Can you work these out from the model? Positions are in its coordinate system, mm. Face numbers are marked on the shaded views. A direction names the side the tool comes from. Coordinates: 2 decimals unless noted, no trailing zeros. Write each loop counter-clockwise with the first axis right and the second up, starting at its lowest first coordinate (ties: lowest second). Pieces come first, ordered by that corner, then holes. Notation, with made-up numbers: (-29.5, 63) - (-4.5, 63) arc R25 cw to (-4.5, 95) - close; hole circle Ø2 at (17, 69.5). An arc over 180 degrees is marked (long way). Write each question's results on one line, items separated by ' | '. Start each with the question number.
```python
from build123d import *

# Parameters (mm, degrees)
BASE_PROFILE_SKETCH_R       = 12.5
BASE_PROFILE_SKETCH_R_2     = 7.5
BASE_PLATE_DEPTH            = 15
SKETCH1_3_W                 = 30
SKETCH1_3_H                 = 15
LOWER_LUG_DEPTH             = 45
LOWER_LUG_CUT_SKETCH_R      = 6
LOWER_LUG_PROFILE_CUT_DEPTH = 45
UPRIGHT_LUG_SKETCH_R        = 6
UPRIGHT_LUG_12_HOLE_DEPTH   = 15


with BuildPart() as part:
    # Base Profile Sketch → Base Plate (new body)
    with BuildSketch(Plane(origin=(0, 0, 0), x_dir=(1, 0, 0), z_dir=(0, 1, 0))):
        with BuildLine():
            Line((150, 25), (0, 25))
            ThreePointArc((0, 25), (-25, 0), (0, -25))
            Line((0, -25), (102.111825559, -25))
            Line((102.111825559, -25), (120, -25))
            Line((120, -25), (150, -25))
            Line((150, -25), (150, 25))
        make_face()
        with Locations(Location((0, 0, 0), (0, 0, 270))):
            Circle(BASE_PROFILE_SKETCH_R, mode=Mode.SUBTRACT)
        with Locations(Location((135, 0, 0), (0, 0, 270))):
            Circle(BASE_PROFILE_SKETCH_R_2, mode=Mode.SUBTRACT)
    extrude(amount=-BASE_PLATE_DEPTH)

    # Sketch1_3 → Lower Lug (add)
    with BuildSketch(Plane(origin=(0, 0, 0), x_dir=(1, 0, 0), z_dir=(0, 1, 0))):
        with Locations((135, -32.5)):
            Rectangle(SKETCH1_3_W, SKETCH1_3_H)
    extrude(amount=-LOWER_LUG_DEPTH)

    # Lower Lug Cut Sketch → Lower Lug Profile Cut (cut)
    with BuildSketch(Plane.XY.offset(40)):
        with Locations((135, -30)):
            Circle(LOWER_LUG_CUT_SKETCH_R)
        with BuildLine():
            Line((120, -54.887951231), (153.351111221, -54.269822589))
            Line((153.351111221, -54.269822589), (153.351111221, -31.584501417))
            Line((153.351111221, -31.584501417), (150, -30))
            ThreePointArc((150, -30), (135, -45), (120, -30))
            Line((120, -30), (109.958480534, -30))
            Line((109.958480534, -30), (120, -54.887951231))
        make_face()
    extrude(amount=-LOWER_LUG_PROFILE_CUT_DEPTH, mode=Mode.SUBTRACT)

    # Upright Lug Sketch → Upright Lug _12 Hole (add)
    with BuildSketch(Plane.XY.offset(25)):
        with BuildLine():
            Line((20, 15), (20, -3.361922894))
            Line((20, -3.361922894), (50, -3.361922894))
            Line((50, -3.361922894), (50, 15))
            ThreePointArc((50, 15), (35, 30), (20, 15))
        make_face()
        with Locations((35, 15)):
            Circle(UPRIGHT_LUG_SKETCH_R, mode=Mode.SUBTRACT)
    extrude(amount=-UPRIGHT_LUG_12_HOLE_DEPTH)


solid = part.part
```
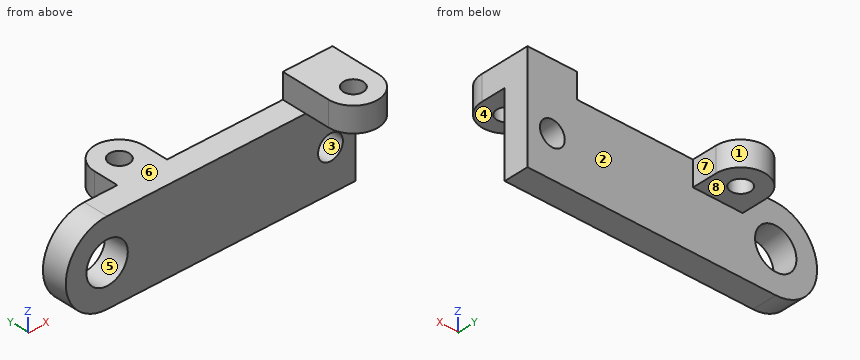
Q1. If we section it at B-B (z = 0): Please give me the cut outline in (x, y), then the cut area to 4 significant figures.
Q2. For the marked faces 4, 5, 6, 7 and 8, which set-ups out of +Z, -Z, +X, -X, +Y, -Y let a thin tool reach every point of the face, with its end or its side?
Q3. I need wall thicknesses on line 1 along X through (y, z) = (-10, 0); line 2 along Y through (x, z) = (35, 20); line 3 along X through (y, z) = (-3.5, 5). Which ranges of each line are inside material? Lowest first, please. Write a range as from..to.
Q4. If we section it at D-D (x = 135): Please give me the cut outline in (y, z), then the cut area to 3 significant figures.
Q5. I'm going to push flat-ended pins straight in: pin 1 Ø12 at (x, z) = (68, 26) entering from +Y; pin 2 Ø13.5 at (x, z) = (135, 0) entering from -Y; pin 3 Ø7.5 at (y, z) = (7, 20) entering from -X; pin 4 Ø15 at (x, y) = (130, -36) entering from -Z. Where does each tip first touch, or does it pass through?
Q6. If we section it at C-C (y = -3.5): Please give me the cut outline in (x, z).
Q7. If we section it at A-A (x = 35): Please give me the cut outline in (y, z), then the cut area to 3 significant figures.
Q8. Thinking about a two-plate mould opening in X: for the marked faces 1, 2 and 3, which applies, pulls with the +X half, pulls with the -X half, needs draft (parallel to the pull), parting line crosses it, or undercut?
Answer list:
1) outline: (-25, -15) - (-12.5, -15) - (-12.5, 0) - (-25, 0) - close; (12.5, -15) - (127.5, -15) - (127.5, 0) - (12.5, 0) - close; (142.5, -15) - (150, -15) - (150, 0) - (142.5, 0) - close | area: 2,025 mm2
2) face 4: -Z, +X, -X, -Y | face 5: +Y, -Y | face 6: +Z, -X, +Y, -Y | face 7: +Z, -Z, +X, +Y | face 8: -Z, +X, -X, +Y
3) line 1: x = -25..-12.5, 12.5..127.5, 142.5..150 | line 2: y = -15..9, 21..30 | line 3: x = -24.49..-11.46, 11.46..129.41, 140.59..150
4) outline: (-45, 25) - (-36, 25) - (-36, 40) - (-45, 40) - close; (-24, 25) - (-15, 25) - (-15, 7.5) - (0, 7.5) - (0, 40) - (-24, 40) - close; (-15, -25) - (0, -25) - (0, -7.5) - (-15, -7.5) - close | area: 1,020 mm2
5) pin 1: stops at y = 0 | pin 2: passes through | pin 3: stops at x = 20 | pin 4: stops at z = 25
6) outline: (0, -25) - (150, -25) - (150, 40) - (120, 40) - (120, 25) - (0, 25) arc R25 ccw to start; hole circle Ø25 at (0, 0); hole circle Ø15 at (135, 0)
7) outline: (-15, -25) - (0, -25) - (0, 10) - (9, 10) - (9, 25) - (-15, 25) - close; (21, 10) - (30, 10) - (30, 25) - (21, 25) - close | area: 1,020 mm2
8) face 1: parting line crosses it | face 2: needs draft | face 3: undercut
